Work out the finished part from the listing and answer in its coordinate system (mm). A direction names the side the tool comes from. Coordinates: 2 decimals unless noted, no trailing zeros. Order: outer loops, then holes, each group sorted by start corner. A loop starts at its lowest first (then second) coordinate and runs counter-clockwise, first axis right, second up. Notation, with made-up numbers: (1.5, 89) - (29.5, 89) arc R24 cw to (29.5, 128) - close; hole circle Ø9 at (10, 6.5). An arc over 180 degrees is marked (long way). Answer as a JSON object with one key per item and string values. Group by question number.
1) Section B-B (x = -10) is taken. Give the vertices of the cut face in (y, z), plus the area to 3 significant figures.
2) Find the intervals of material crossed by line 1 along Z through (x, y) = (-42.5, 13); line 2 along Y through (x, z) = (-5.5, 2); line 3 along Z through (x, y) = (-12.5, 33.5), in increasing order.
3) A tool of negligible diameter and unlimited length cuts with its end or side. For faces 4 (the face through (-7.1, 70.92, 50.83)), 5 (the face through (-16, 48, 32)), 6 (the face through (-34, 15, -2)), 7 (the face through (-22.5, 33.8, -44.8)), from which of +Z, -Z, +X, -X, +Y, -Y can it reach the whole face along a straight path? Write none if from no direction.
4) The mould has two halves that part along Z. Classify faces 1 (the face through (-50.58, 5.07, -2.76)), 2 (the face through (-37, 46, -52)), 3 (the face through (-24, 30, -70)): released by +Z, released by -Z, zero draft, split by the parting line, or undercut.
5) Each of these flat-tipped pins is pushed along its axis until it touches: P1, Ø17.5, axis at x = -47.5, z = -3, coming from the +Y side; P2, Ø4, axis at x = -16.5, y = 45.5, coming from the +Z side; P3, Ø8, axis at y = 15.5, z = -1.5, coming from the -X side; P4, Ø9.5, axis at x = -44.72, z = -1.46, coming from the +Y side. Where does it stop, or does it pass through?
6) Section A-A (z = 51) is taken. Give the vertices of the cut face in (x, y), plus the area to 3 significant figures.
7) Section C-C (y = 59) is taken. Give the vertices of the cut face in (x, z).
8) Section D-D (y = 5) is taken. Give the vertices of the cut face in (x, z), plus the area to 3 significant figures.
from build123d import *

# Parameters (mm, degrees)
BASE_ANGLE_BODY_DEPTH        = 70
FRONT_EDGE_RELIEF_CUT_DEPTH  = 118.524465538
LONG_EDGE_RELIEF_CUT_DEPTH   = 140
REAR_STEP_PAD_SKETCH_W       = 102
REAR_STEP_PAD_SKETCH_H       = 56
REAR_STEP_PAD_DEPTH          = 5
UPRIGHT_SLOT_CUT_DEPTH       = 112.534747949
PAD_RELIEF_SKETCH_R          = 9
PAD_RELIEF_CUT_DEPTH         = 110.749715262
REAR_BLOCK_SKETCH_W          = 37
REAR_BLOCK_SKETCH_H          = 26
REAR_BLOCK_DEPTH             = 36
REAR_POCKET_SKETCH_W         = 30
REAR_POCKET_SKETCH_H         = 10
REAR_POCKET_CUT_DEPTH        = 22
UPRIGHT_HOLE_SKETCH_R        = 6
UPRIGHT_HOLE_CUT_DEPTH       = 22
REAR_BLOCK_PROFILE_CUT_DEPTH = 22


with BuildPart() as part:
    # Base Angle Profile Sketch → Base Angle Body (new, symmetric)
    with BuildSketch(Plane.XY):
        Polygon((0, 0), (-56, 0), (-56, 20), (-14, 20), (-14, 76), (0, 76), align=None)
    extrude(amount=BASE_ANGLE_BODY_DEPTH, both=True)

    # Front Edge Relief Sketch → Front Edge Relief Cut (cut, through all)
    with BuildSketch(Plane(origin=(0, 76, 0), x_dir=(1, 0, 0), z_dir=(0, 1, 0))):
        with BuildLine():
            Line((-5, 70), (0, 70))
            Line((0, 70), (0, 65))
            ThreePointArc((0, 65), (-1.464466094, 68.535533906), (-5, 70))
        make_face()
        with BuildLine():
            Line((0, -70), (0, -65))
            ThreePointArc((0, -65), (-1.464466094, -68.535533906), (-5, -70))
            Line((-5, -70), (0, -70))
        make_face()
    extrude(amount=-FRONT_EDGE_RELIEF_CUT_DEPTH, mode=Mode.SUBTRACT)

    # Long Edge Relief Sketch → Long Edge Relief Cut (cut)
    with BuildSketch(Plane(origin=(0, 20, 0), x_dir=(1, 0, 0), z_dir=(0, 1, 0))):
        with BuildLine():
            Line((-56, -65), (-56, -70))
            Line((-56, -70), (-51, -70))
            ThreePointArc((-51, -70), (-54.535533906, -68.535533906), (-56, -65))
        make_face()
    extrude(amount=-LONG_EDGE_RELIEF_CUT_DEPTH, mode=Mode.SUBTRACT)

    # Rear Step Pad Sketch → Rear Step Pad (add)
    with BuildSketch(Plane.ZY.offset(14)):
        with Locations((-19, 48)):
            Rectangle(REAR_STEP_PAD_SKETCH_W, REAR_STEP_PAD_SKETCH_H)
    extrude(amount=REAR_STEP_PAD_DEPTH)

    # Upright Slot Sketch → Upright Slot Cut (cut, through all)
    with BuildSketch(Plane.ZY.offset(14)):
        with BuildLine():
            Line((43.076503739, 33), (43.076503739, 63))
            ThreePointArc((43.076503739, 63), (51, 70.923496261), (58.923496261, 63))
            Line((58.923496261, 63), (58.923496261, 33))
            ThreePointArc((58.923496261, 33), (51, 25.076503739), (43.076503739, 33))
        make_face()
    extrude(amount=-UPRIGHT_SLOT_CUT_DEPTH, mode=Mode.SUBTRACT)

    # Pad Relief Sketch → Pad Relief Cut (cut, through all)
    with BuildSketch(Plane.ZY.offset(19)):
        with Locations((2, 59)):
            Circle(PAD_RELIEF_SKETCH_R)
    extrude(amount=-PAD_RELIEF_CUT_DEPTH, mode=Mode.SUBTRACT)

    # Rear Block Sketch → Rear Block (add)
    with BuildSketch(Plane(origin=(0, 0, -70), x_dir=(-1, 0, 0), z_dir=(0, 0, -1))):
        with Locations((37.5, 33)):
            Rectangle(REAR_BLOCK_SKETCH_W, REAR_BLOCK_SKETCH_H)
    extrude(amount=-REAR_BLOCK_DEPTH)

    # Rear Pocket Sketch → Rear Pocket Cut (cut)
    with BuildSketch(Plane.ZY.offset(56)):
        with Locations((-1.461655613, 15)):
            Rectangle(REAR_POCKET_SKETCH_W, REAR_POCKET_SKETCH_H)
    extrude(amount=-REAR_POCKET_CUT_DEPTH, mode=Mode.SUBTRACT)

    # Upright Hole Sketch → Upright Hole Cut (cut)
    with BuildSketch(Plane(origin=(0, 10, 0), x_dir=(1, 0, 0), z_dir=(0, 1, 0))):
        with Locations(Location((-44.72410092, 1.461655613, 0), (0, 0, 270))):
            Circle(UPRIGHT_HOLE_SKETCH_R)
    extrude(amount=-UPRIGHT_HOLE_CUT_DEPTH, mode=Mode.SUBTRACT)

    # Rear Block Profile Sketch → Rear Block Profile Cut (cut)
    with BuildSketch(Plane.XY.offset(-34)):
        with BuildLine():
            Line((-45.5, 39.678271728), (-28.5, 39.678271728))
            ThreePointArc((-28.5, 39.678271728), (-22.5, 33.678271728), (-28.5, 27.678271728))
            Line((-28.5, 27.678271728), (-45.5, 27.678271728))
            ThreePointArc((-45.5, 27.678271728), (-51.5, 33.678271728), (-45.5, 39.678271728))
        make_face()
    extrude(amount=-REAR_BLOCK_PROFILE_CUT_DEPTH, mode=Mode.SUBTRACT)


solid = part.part
Report:
{
 "1": {"outline": "(0, -70) - (76, -70) - (76, 70) - (0, 70) - close; hole (33, 43.08) - (63, 43.08) arc R7.92 ccw to (63, 58.92) - (33, 58.92) arc R7.92 ccw to start; hole circle Ø18 at (59, 2)", "area": "9,710 mm²"},
 "2": {"line 1": "z = -70 to -16.46, 13.54 to 70", "line 2": "y = 0 to 50, 68 to 76", "line 3": "z = -70 to 43.08, 58.92 to 70"},
 "3": {"face 4": "+X, -X", "face 5": "+Z, -X, +Y", "face 6": "-X, +Y", "face 7": "+Z"},
 "4": {"face 1": "undercut", "face 2": "zero draft", "face 3": "released by -Z"},
 "5": {"P1": "stops at y = 10", "P2": "stops at z = 32", "P3": "stops at x = -34", "P4": "passes through"},
 "6": {"outline": "(-56, 0) - (0, 0) - (0, 25.08) - (-14, 25.08) - (-14, 20) - (-56, 20) - close; (-14, 70.92) - (0, 70.92) - (0, 76) - (-14, 76) - close", "area": "1,260 mm²"},
 "7": {"outline": "(-19, -70) - (-5, -70) arc R5 ccw to (0, -65) - (0, -7) - (-19, -7) - close; (-19, 11) - (0, 11) - (0, 43.08) - (-14, 43.08) - (-14, 32) - (-19, 32) - close; (-14, 58.92) - (0, 58.92) - (0, 65) arc R5 ccw to (-5, 70) - (-14, 70) - close"},
 "8": {"outline": "(-56, -70) - (-5, -70) arc R5 ccw to (0, -65) - (0, 65) arc R5 ccw to (-5, 70) - (-51, 70) arc R5 ccw to (-56, 65) - close; hole circle Ø12 at (-44.72, -1.46)", "area": "7,710 mm²"}
}
